```python
from build123d import *

# Parameters (mm, degrees)
SKETCH1_W          = 4.5
SKETCH1_H          = 27
CUT_EXTRUDE1_DEPTH = 15


with BuildPart() as part:
    # Sketch1 → Revolve3 (revolve)
    with BuildSketch(Plane(origin=(0, 0, 0), x_dir=(1, 0, 0), z_dir=(0, 1, 0)), mode=Mode.PRIVATE) as revolve3_sk:
        with Locations((2.25, 0)):
            Rectangle(SKETCH1_W, SKETCH1_H)
        Polygon((0, -13.5), (4.5, -13.5), (0, -16), align=None)
        Polygon((9, 16.5), (4.5, 13.5), (0, 13.5), (0, 16.5), align=None)
    revolve(revolve3_sk.sketch.rotate(Axis((0, 0, -13.5), (0, 0, 1)), 180), axis=Axis((0, 0, -13.5), (0, 0, 1)))

    # Sketch2 → Cut-Extrude1 (cut, symmetric)
    with BuildSketch(Plane(origin=(0, 0, 0), x_dir=(1, 0, 0), z_dir=(0, 1, 0))):
        Polygon((0, 16.5), (0.75, 16.5), (0.75, 15), (-0.75, 15), (-0.75, 16.5), align=None)
    extrude(amount=CUT_EXTRUDE1_DEPTH, both=True, mode=Mode.SUBTRACT)


solid = part.part
```
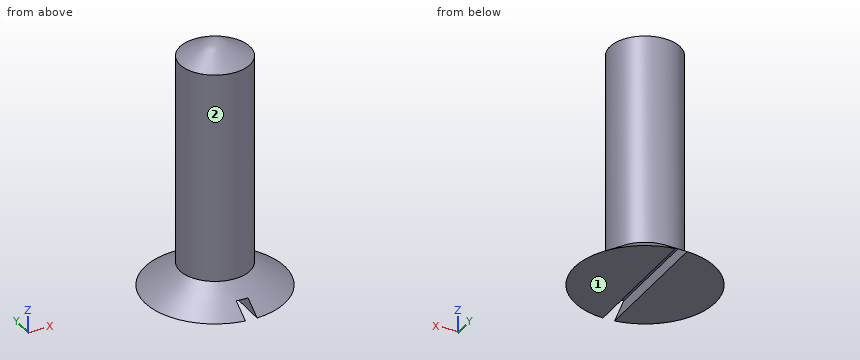
Model file for the job. Use its own axes, mm. Face numbers are marked on the shaded views. A direction names the side the tool comes from. Coordinates: 2 decimals unless noted, no trailing zeros. Loops run counter-clockwise (first coordinate to the right, second up) from the corner with the lowest first, then second, coordinate; pieces in that order, holes last. Notation, with made-up numbers: (79, -38) - (113, -38) arc R27 cw to (113, -14) - close; hole circle Ø11 at (23, 22.25). An arc over 180 degrees is marked (long way). Answer as a JSON object with one key per item and string values. Group by question number.
(1) Tool access for the marked faces 1 and 2: list every direction of +Z, -Z, +X, -X, +Y, -Y with a clear straight run to the whole face (end or side of a thin tool).
(2) Cut at A-A (z = 0). Give the cut face in (x, y), then the cut area to 3 significant figures.
(3) Probe line 1 along X through (y, z) = (-0.25, -4); line 2 along Z through (x, y) = (4, 2.5); line 3 along Y through (x, z) = (-2, -14). List the from-to ranges inside material, lowest first.
(4) Flat gauge pins, fed straight in: pin 1 (1.5 mm diameter, centred on x = -4.5, y = 3, fed in from +Z); pin 2 (1.2 mm diameter, centred on y = -2, z = -15.5, fed in from +X); pin 3 (0.8 mm diameter, centred on x = 0, y = -0.5, fed in from -Z). Where does each tip first touch, or does it go through?
Geometry says:
{
 "1": {"face 1": "-Z, +X, -X, +Y, -Y", "face 2": "+Z"},
 "2": {"outline": "circle Ø9 at (0, 0)", "area": "63.6 mm^2"},
 "3": {"line 1": "x = -4.49 to 4.49", "line 2": "z = -16.5 to -13.64", "line 3": "y = -4.85 to 4.85"},
 "4": {"pin 1": "stops at z = -13.61", "pin 2": "stops at x = 8.17", "pin 3": "stops at z = -15"}
}
